Design review of the part built by this model. Coordinates are the model's own, in mm. Coordinates: 2 decimals unless noted, no trailing zeros. Loops run counter-clockwise (first coordinate to the right, second up) from the corner with the lowest first, then second, coordinate; pieces in that order, holes last.
Q1. Wall thickness on probe 1 along Y at (x, z) = (-36, 5): over which ranges is the line inside the solid? List them lowest first.
Q2. Draft analysis for pull direction Y (two halves, no side actions). For faces 1 (the face through (-44.848, 32.389, 6.858)), 2 (the face through (-1, 0, 0)), 3 (the face through (-34.66, 29.11, 3.55)), state which applies: released by +Y, released by -Y, zero draft, split by the parting line, or undercut.
Q3. Add section B-B on x = 36. Give the boundary of the cut face in (y, z).
Q4. Add section A-A on y = -27. Give the boundary of the cut face in (x, z).
```python
from build123d import *

# Parameters (mm, degrees)
SKETCH_1_W                  = 92
SKETCH_1_H                  = 67
EXTRUDE_1_DEPTH             = 7
FILLET_1_R                  = 3
SKETCH_2_R                  = 2.5
CUT_EXTRUDE_1_DEPTH         = 10
PATTERN_LINEAR_1_COUNT      = 2
PATTERN_LINEAR_1_PITCH      = 72
PATTERN_LINEAR_1_COUNT_DIR2 = 2
PATTERN_LINEAR_1_PITCH_DIR2 = 54
CHAMFER_1_SIZE              = 0.5


with BuildPart() as part:
    # 草图1 → 凸台-拉伸1 (new body)
    with BuildSketch(Plane.XY):
        Rectangle(SKETCH_1_W, SKETCH_1_H)
    extrude(amount=EXTRUDE_1_DEPTH)

    # 圆角1
    fillet_1_edges = [part.edges().sort_by_distance(p)[0] for p in [
        (46, -33.5, 3.5),
        (-46, -33.5, 3.5),
        (-46, 33.5, 3.5),
        (46, 33.5, 3.5),
    ]]
    fillet(fillet_1_edges, radius=FILLET_1_R)

    # 草图2 → 切除-拉伸1 (cut)
    with BuildSketch(Plane.XY.offset(7)):
        with Locations((-36, 27)):
            Circle(SKETCH_2_R)
    cut_extrude_1 = extrude(amount=-CUT_EXTRUDE_1_DEPTH, mode=Mode.SUBTRACT)

    # 阵列(线性)1: Cut-Extrude 1 2 × 2
    with Locations(*[(i * PATTERN_LINEAR_1_PITCH, -j * PATTERN_LINEAR_1_PITCH_DIR2, 0) for i in range(PATTERN_LINEAR_1_COUNT) for j in range(PATTERN_LINEAR_1_COUNT_DIR2) if (i, j) != (0, 0)]):
        add(cut_extrude_1, mode=Mode.SUBTRACT)

    # 倒角1
    chamfer_1_edges = [part.edges().sort_by_distance(p)[0] for p in [
        (46, 0, 0),
        (46, 0, 7),
        (0, -33.5, 0),
        (-46, 0, 0),
        (0, 33.5, 0),
        (-45.121320344, 32.621320344, 0),
        (45.121320344, 32.621320344, 0),
        (-45.121320344, -32.621320344, 0),
        (45.121320344, -32.621320344, 0),
        (0, -33.5, 7),
        (0, 33.5, 7),
        (-46, 0, 7),
        (-45.121320344, 32.621320344, 7),
        (45.121320344, 32.621320344, 7),
        (-45.121320344, -32.621320344, 7),
        (45.121320344, -32.621320344, 7),
    ]]
    chamfer(chamfer_1_edges, length=CHAMFER_1_SIZE)


solid = part.part
```
Entries:
1. probe 1: y = -33.5 to -29.5, -24.5 to 24.5, 29.5 to 33.5
2. face 1: released by +Y
2. face 2: zero draft
2. face 3: undercut
3. outline: (-33.5, 0.5) - (-33, 0) - (-29.5, 0) - (-29.5, 7) - (-33, 7) - (-33.5, 6.5) - close; (-24.5, 0) - (24.5, 0) - (24.5, 7) - (-24.5, 7) - close; (29.5, 0) - (33, 0) - (33.5, 0.5) - (33.5, 6.5) - (33, 7) - (29.5, 7) - close
4. outline: (-46, 0.5) - (-45.5, 0) - (-38.5, 0) - (-38.5, 7) - (-45.5, 7) - (-46, 6.5) - close; (-33.5, 0) - (33.5, 0) - (33.5, 7) - (-33.5, 7) - close; (38.5, 0) - (45.5, 0) - (46, 0.5) - (46, 6.5) - (45.5, 7) - (38.5, 7) - close
